Part print with two shaded views. Sizes in mm from the minimum x, y, z corner. A direction names the side the tool comes from. Coordinates: 2 decimals unless noted, no trailing zeros. Write each loop counter-clockwise with the first axis right and the second up, starting at its lowest first coordinate (ties: lowest second). Pieces come first, ordered by that corner, then holes. Notation, with made-up numbers: M 35,24.25 L 40,24.25 A16 cw 40,33.25 Z; hole C 19.25,27 d3. An arc over 180 degrees is marked long. Answer in a Markdown table with one row per item. Add a question column.
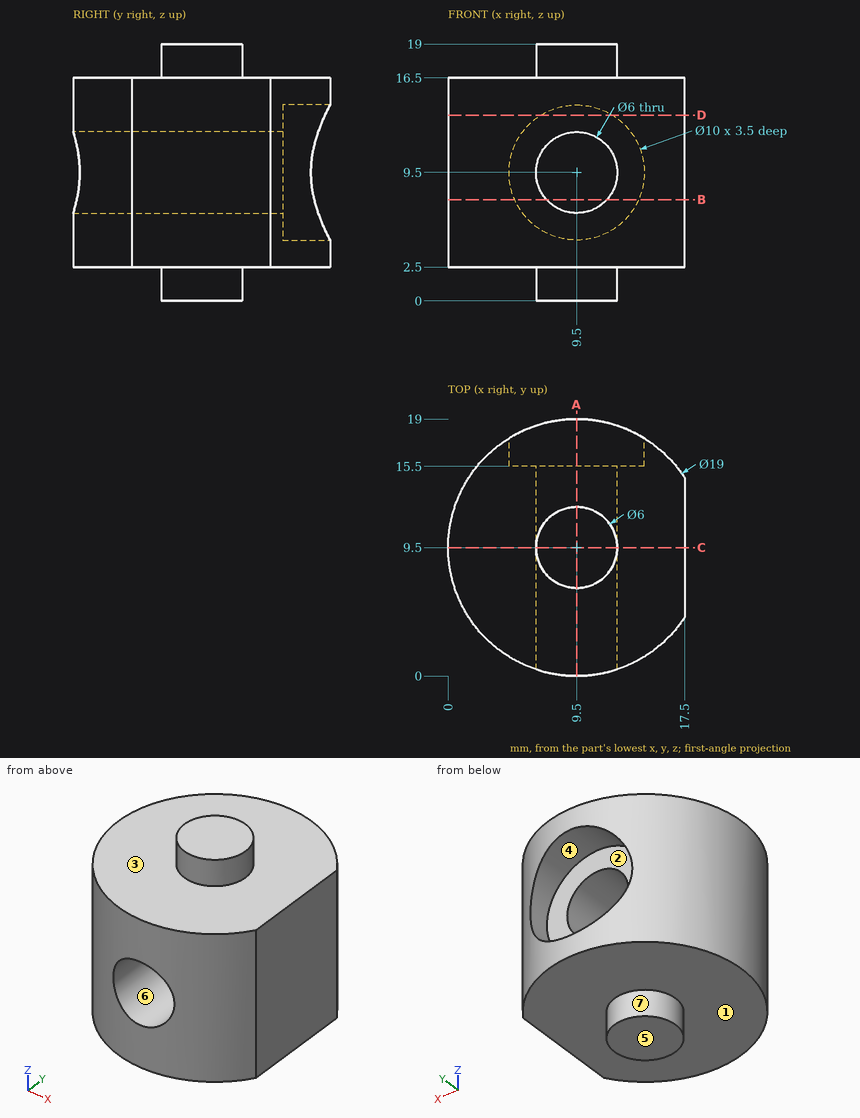
1) Which spindle directions (+Z, -Z, +X, -X, +Y, -Y) get a long thin tool onto all of the face, cutting with end or side? Do the marked faces 1, 2 and 3. Say none if no direction does.
2) Slice it at D-D (z = 13.75). Give the cut face in (x, y), then the cut area to 3 significant figures.
3) Flat gauge pin, fed straight in: pin 1 Ø8 at (x, y) = (2.5, 5) entering from +Z. Where does the tip first touch, or does it go through?
4) Drill centre lines: probe 1 along Z at (x, y) = (3.5, 13.5); probe 2 along X at (y, z) = (12.75, 12.25); probe 3 along X at (y, z) = (6.5, 10.75). Where is each one in solid material? Low to high.
5) Slice it at A-A (x = 9.5). Give the cut face in (y, z).
6) Two-plate mould, pull along Z, no slides. Class the marked faces 4, 5, 6 and 7: released by +Z, released by -Z, zero draft, split by the parting line, or undercut.
7) Slice it at B-B (z = 7.5). Give the cut face in (x, y).
8) Slice it at C-C (y = 9.5). Give the cut face in (x, z).
Ans:
| question | item | result |
|---|---|---|
| 1 | face 1 | -Z |
| 1 | face 2 | +Y |
| 1 | face 3 | +Z |
| 2 | outline | M 6.87,15.5 L 6.87,18.63 A9.5 ccw long 17.5,4.38 L 17.5,14.62 A9.5 ccw 12.13,18.63 L 12.13,15.5 Z |
| 2 | area | 255 mm2 |
| 3 | pin 1 | stops at z = 16.5 |
| 4 | probe 1 | z = 2.5 to 16.5 |
| 4 | probe 2 | x = 0.57 to 8.3, 10.7 to 17.5 |
| 4 | probe 3 | x = 0.49 to 6.77, 12.23 to 17.5 |
| 5 | outline | M 0,2.5 L 6.5,2.5 L 6.5,0 L 12.5,0 L 12.5,2.5 L 19,2.5 L 19,4.5 L 15.5,4.5 L 15.5,6.5 L 0,6.5 Z; M 0,12.5 L 15.5,12.5 L 15.5,14.5 L 19,14.5 L 19,16.5 L 12.5,16.5 L 12.5,19 L 6.5,19 L 6.5,16.5 L 0,16.5 Z |
| 6 | face 4 | undercut |
| 6 | face 5 | released by -Z |
| 6 | face 6 | undercut |
| 6 | face 7 | zero draft |
| 7 | outline | M 4.92,15.5 L 4.92,17.82 A9.5 ccw 7.26,0.27 L 7.26,15.5 Z; M 11.74,0.27 A9.5 ccw 17.5,4.38 L 17.5,14.62 A9.5 ccw 14.08,17.82 L 14.08,15.5 L 11.74,15.5 Z |
| 8 | outline | M 0,2.5 L 6.5,2.5 L 6.5,0 L 12.5,0 L 12.5,2.5 L 17.5,2.5 L 17.5,16.5 L 12.5,16.5 L 12.5,19 L 6.5,19 L 6.5,16.5 L 0,16.5 Z; hole C 9.5,9.5 d6 |
